For this review, take the finished solid that the model builds, in its own axes (mm). Face numbers are marked on the shaded views. A direction names the side the tool comes from. Round coordinates to 2 decimals unless told otherwise and drop trailing zeros. Loops run counter-clockwise (first coordinate to the right, second up) from the corner with the lowest first, then second, coordinate; pieces in that order, holes last.
1. Clearance check with flat-ended pins moving along their axes: pin 1 Ø1.5 at (x, z) = (-43.5, 35) entering from +Y; pin 2 Ø6 at (x, z) = (-10, 105.5) entering from +Y; pin 3 Ø8 at (y, z) = (-6, 108.5) entering from +X. State where each tip first meets the part, or that it passes through.
2. Consider section C-C on z = 13. State the section outline as (x, y) points.
3. To check wall thickness, follow line 1 along Y through (x, z) = (0, 20.25); line 2 along Z through (x, y) = (25, -48); line 3 along Z through (x, y) = (47.5, 32). State the ranges of each line that lie inside material, in increasing order.
4. Consider section B-B on x = 40. State the section outline as (y, z) points.
5. Consider section D-D on x = -25. State the section outline as (y, z) points.
6. Consider section A-A on y = 9. State the section outline as (x, z) points, then the cut area to 3 significant figures.
7. Draft analysis for pull direction X (two halves, no side actions). For the marked faces 1, 2 and 3, state which applies: released by +X, released by -X, zero draft, split by the parting line, or undercut.
8. Tool access review of the marked faces 4, 5, 6, 7 and 8: name each direction out of +Z, -Z, +X, -X, +Y, -Y from which nothing blocks a thin tool from reaching the whole face with its end or side.
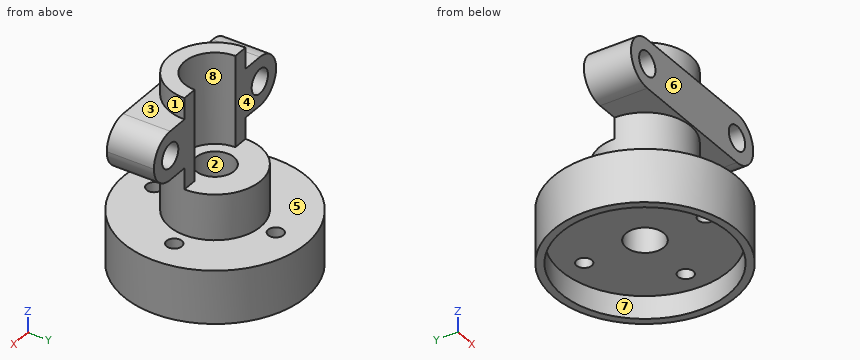
from build123d import *

# Parameters (mm, degrees)
BASE_FLANGE_SKETCH_R              = 60
BASE_FLANGE_SKETCH_R_2            = 55
BASE_FLANGE_PLATE_DEPTH           = 15
ROUND_FLANGE_SKETCH_120_R         = 60
ROUND_FLANGE_120_DEPTH            = 20
FLANGE_BOLT_HOLES_SKETCH_R        = 5
FLANGE_BOLT_HOLES_4X_10_DEPTH     = 20
HUB_BOSS_SKETCH_R                 = 30
HUB_BOSS_SKETCH_R_2               = 12.5
HUB_BOSS_DEPTH                    = 30
HUB_START                         = -30
HUB_BORE_SKETCH_25_R              = 12.5
HUB_BORE_25_DEPTH                 = 30
CRADLE_BODY_DEPTH                 = 60
CRADLE_LUGS_SKETCH_R              = 16
CRADLE_LUGS_SKETCH_R_2            = 8
CRADLE_MOUNTING_LUGS_DEPTH        = 31
CRADLE_BORE_SKETCH_40_R           = 20
CRADLE_BORE_40_DEPTH              = 60
LUG_PAD_SKETCH_R                  = 8
LUG_PADS_DEPTH                    = 32
PARTING_SLOT_SKETCH_W             = 120
PARTING_SLOT_SKETCH_H             = 1
CRADLE_PARTING_SLOT_1MM_DEPTH     = 32
LUG_BORE_SKETCH_40_R              = 20
CRADLE_BORE_40_THROUGH_LUGS_DEPTH = 60


with BuildPart() as part:
    # Base Flange Sketch → Base Flange Plate (new body)
    with BuildSketch(Plane.XY):
        Circle(BASE_FLANGE_SKETCH_R)
        Circle(BASE_FLANGE_SKETCH_R_2, mode=Mode.SUBTRACT)
    extrude(amount=BASE_FLANGE_PLATE_DEPTH)

    # Round Flange Sketch Ø120 → Round Flange Ø120 (add)
    with BuildSketch(Plane.XY.offset(15)):
        Circle(ROUND_FLANGE_SKETCH_120_R)
    extrude(amount=ROUND_FLANGE_120_DEPTH)

    # Flange Bolt Holes Sketch → Flange Bolt Holes 4xØ10 (cut)
    with BuildSketch(Plane.XY.offset(35)):
        with Locations((0, 40)):
            Circle(FLANGE_BOLT_HOLES_SKETCH_R)
        with Locations((40, 0)):
            Circle(FLANGE_BOLT_HOLES_SKETCH_R)
        with Locations((0, -40)):
            Circle(FLANGE_BOLT_HOLES_SKETCH_R)
        with Locations((-40, 0)):
            Circle(FLANGE_BOLT_HOLES_SKETCH_R)
    extrude(amount=-FLANGE_BOLT_HOLES_4X_10_DEPTH, mode=Mode.SUBTRACT)

    # Hub Boss Sketch → Hub Boss (add)
    with BuildSketch(Plane.XY.offset(35)):
        Circle(HUB_BOSS_SKETCH_R)
        Circle(HUB_BOSS_SKETCH_R_2, mode=Mode.SUBTRACT)
    extrude(amount=HUB_BOSS_DEPTH)

    # Hub Bore Sketch Ø25 → Hub Bore Ø25 (cut)
    with BuildSketch(Plane.XY.offset(35).offset(HUB_START)):
        Circle(HUB_BORE_SKETCH_25_R)
    extrude(amount=HUB_BORE_25_DEPTH, mode=Mode.SUBTRACT)

    # Cradle Body Sketch → Cradle Body (add)
    with BuildSketch(Plane.XY.offset(65)):
        with BuildLine():
            Line((-30, 0), (-12.5, 0))
            ThreePointArc((-12.5, 0), (0, -12.5), (12.5, 0))
            Line((12.5, 0), (30, 0))
            ThreePointArc((30, 0), (0, -30), (-30, 0))
        make_face()
    extrude(amount=CRADLE_BODY_DEPTH)


with BuildPart() as body_2:
    # Cradle Lugs Sketch → Cradle Mounting Lugs (new body)
    # profile 1 of 6: a face of its own
    with BuildSketch(Plane(origin=(0, 0, 0), x_dir=(1, 0, 0), z_dir=(0, 1, 0))):
        with Locations((-44, -95)):
            Circle(CRADLE_LUGS_SKETCH_R)
        with Locations(Location((-44, -95, 0), (0, 0, 270))):
            Circle(CRADLE_LUGS_SKETCH_R_2, mode=Mode.SUBTRACT)
    # profile 2 of 6: a face of its own
    with BuildSketch(Plane(origin=(0, 0, 0), x_dir=(1, 0, 0), z_dir=(0, 1, 0))):
        with BuildLine():
            Line((-12.5, -79), (-44, -79))
            ThreePointArc((-44, -79), (-32.686291501, -83.686291501), (-28, -95))
            ThreePointArc((-28, -95), (-32.686291501, -106.313708499), (-44, -111))
            Line((-44, -111), (-12.5, -111))
            Line((-12.5, -111), (12.5, -111))
            Line((12.5, -111), (12.5, -79))
            Line((12.5, -79), (-12.5, -79))
        make_face()
    # profile 3 of 6: a face of its own
    with BuildSketch(Plane(origin=(0, 0, 0), x_dir=(1, 0, 0), z_dir=(0, 1, 0))):
        with BuildLine():
            Line((30, -79), (12.5, -79))
            Line((12.5, -79), (12.5, -111))
            Line((12.5, -111), (30, -111))
            Line((30, -111), (30, -102.745966692))
            ThreePointArc((30, -102.745966692), (28, -95), (30, -87.254033308))
            Line((30, -87.254033308), (30, -79))
        make_face()
    # profile 4 of 6: a face of its own
    with BuildSketch(Plane(origin=(0, 0, 0), x_dir=(1, 0, 0), z_dir=(0, 1, 0))):
        with BuildLine():
            Line((44, -79), (30, -79))
            Line((30, -79), (30, -87.254033308))
            ThreePointArc((30, -87.254033308), (35.873975975, -81.217121725), (44, -79))
        make_face()
    # profile 5 of 6: a face of its own
    with BuildSketch(Plane(origin=(0, 0, 0), x_dir=(1, 0, 0), z_dir=(0, 1, 0))):
        with BuildLine():
            Line((30, -102.745966692), (30, -111))
            Line((30, -111), (44, -111))
            ThreePointArc((44, -111), (35.873975975, -108.782878275), (30, -102.745966692))
        make_face()
    # profile 6 of 6: a face of its own
    with BuildSketch(Plane(origin=(0, 0, 0), x_dir=(1, 0, 0), z_dir=(0, 1, 0))):
        with BuildLine():
            ThreePointArc((60, -95), (55.313708499, -83.686291501), (44, -79))
            ThreePointArc((44, -79), (35.873975975, -81.217121725), (30, -87.254033308))
            Line((30, -87.254033308), (30, -102.745966692))
            ThreePointArc((30, -102.745966692), (35.873975975, -108.782878275), (44, -111))
            ThreePointArc((44, -111), (55.313708499, -106.313708499), (60, -95))
        make_face()
        with Locations(Location((44, -95, 0), (0, 0, 270))):
            Circle(CRADLE_LUGS_SKETCH_R_2, mode=Mode.SUBTRACT)
    extrude(amount=-CRADLE_MOUNTING_LUGS_DEPTH)


with BuildPart() as cradle_bore_40_tool:
    # Cradle Bore Sketch Ø40 → Cradle Bore Ø40 (new body)
    with BuildSketch(Plane.XY.offset(125)):
        Circle(CRADLE_BORE_SKETCH_40_R)
    extrude(amount=-CRADLE_BORE_40_DEPTH)


with BuildPart() as part_1:
    add(part.part)

    # Cradle Bore Ø40: cut by cradle_bore_40_tool
    add(cradle_bore_40_tool.part, mode=Mode.SUBTRACT)



with BuildPart() as body_2_1:
    add(body_2.part)

    # Cradle Bore Ø40: cut by cradle_bore_40_tool
    add(cradle_bore_40_tool.part, mode=Mode.SUBTRACT)


with BuildPart() as part_2:
    add(part_1.part)

    add(body_2_1.part)  # Lug Pads merges body 2
    # Lug Pad Sketch → Lug Pads (add)
    # profile 1 of 4: a face of its own
    with BuildSketch(Plane.XZ.offset(31)):
        with BuildLine():
            ThreePointArc((-28, 95), (-32.686291501, 106.313708499), (-44, 111))
            ThreePointArc((-44, 111), (-60, 95), (-44, 79))
            ThreePointArc((-44, 79), (-32.686291501, 83.686291501), (-28, 95))
        make_face()
        with Locations(Location((-44, 95, 0), (0, 0, 270))):
            Circle(LUG_PAD_SKETCH_R, mode=Mode.SUBTRACT)
    # profile 2 of 4: a face of its own
    with BuildSketch(Plane.XZ.offset(31)):
        with BuildLine():
            Line((44, 111), (-44, 111))
            ThreePointArc((-44, 111), (-32.686291501, 106.313708499), (-28, 95))
            ThreePointArc((-28, 95), (-32.686291501, 83.686291501), (-44, 79))
            Line((-44, 79), (44, 79))
            ThreePointArc((44, 79), (35.873975975, 81.217121725), (30, 87.254033308))
            ThreePointArc((30, 87.254033308), (28, 95), (30, 102.745966692))
            ThreePointArc((30, 102.745966692), (35.873975975, 108.782878275), (44, 111))
        make_face()
    # profile 3 of 4: a face of its own
    with BuildSketch(Plane.XZ.offset(31)):
        with BuildLine():
            ThreePointArc((30, 87.254033308), (28, 95), (30, 102.745966692))
            Line((30, 102.745966692), (30, 87.254033308))
        make_face()
    # profile 4 of 4: a face of its own
    with BuildSketch(Plane.XZ.offset(31)):
        with BuildLine():
            ThreePointArc((60, 95), (55.313708499, 106.313708499), (44, 111))
            ThreePointArc((44, 111), (35.873975975, 108.782878275), (30, 102.745966692))
            Line((30, 102.745966692), (30, 87.254033308))
            ThreePointArc((30, 87.254033308), (35.873975975, 81.217121725), (44, 79))
            ThreePointArc((44, 79), (55.313708499, 83.686291501), (60, 95))
        make_face()
        with Locations(Location((44, 95, 0), (0, 0, 270))):
            Circle(LUG_PAD_SKETCH_R, mode=Mode.SUBTRACT)
    extrude(amount=-LUG_PADS_DEPTH)

    # Parting Slot Sketch → Cradle Parting Slot 1mm (cut)
    with BuildSketch(Plane.XY.offset(111)):
        with Locations((0, 0.5)):
            Rectangle(PARTING_SLOT_SKETCH_W, PARTING_SLOT_SKETCH_H)
    extrude(amount=-CRADLE_PARTING_SLOT_1MM_DEPTH, mode=Mode.SUBTRACT)

    # Lug Bore Sketch Ø40 → Cradle Bore Ø40 Through Lugs (cut)
    with BuildSketch(Plane.XY.offset(125)):
        Circle(LUG_BORE_SKETCH_40_R)
    extrude(amount=-CRADLE_BORE_40_THROUGH_LUGS_DEPTH, mode=Mode.SUBTRACT)


solid = part_2.part
Resolved:
1. pin 1: stops at y = 42.1
1. pin 2: stops at y = -15.2
1. pin 3: stops at x = 56.87
2. outline: circle Ø120 at (0, 0); hole circle Ø110 at (0, 0)
3. line 1: y = -60 to -45, -35 to -12.5, 12.5 to 35, 45 to 60
3. line 2: z = 15 to 35
3. line 3: z = 0 to 35
4. outline: (-44.72, 0) - (-37.75, 0) - (-37.75, 15) - (-5, 15) - (-5, 35) - (-44.72, 35) - close; (-31, 79) - (0, 79) - (0, 88.07) - (-31, 88.07) - close; (-31, 101.93) - (0, 101.93) - (0, 111) - (-31, 111) - close; (5, 15) - (37.75, 15) - (37.75, 0) - (44.72, 0) - (44.72, 35) - (5, 35) - close
5. outline: (-54.54, 0) - (-48.99, 0) - (-48.99, 15) - (48.99, 15) - (48.99, 0) - (54.54, 0) - (54.54, 35) - (16.58, 35) - (16.58, 65) - (0, 65) - (0, 125) - (-16.58, 125) - (-16.58, 111) - (-31, 111) - (-31, 79) - (-16.58, 79) - (-16.58, 35) - (-54.54, 35) - close
6. outline: (-59.32, 0) - (-54.26, 0) - (-54.26, 15) - (-8.67, 15) - (-8.67, 65) - (-28.62, 65) - (-28.62, 35) - (-59.32, 35) - close; (8.67, 15) - (54.26, 15) - (54.26, 0) - (59.32, 0) - (59.32, 35) - (28.62, 35) - (28.62, 65) - (8.67, 65) - close
6. area: 3,370 mm2
7. face 1: split by the parting line
7. face 2: undercut
7. face 3: zero draft
8. face 4: +Z, +X, -X, +Y
8. face 5: none
8. face 6: +Z, +X, -X, -Y
8. face 7: -Z
8. face 8: +Z, +Y
